```python
from build123d import *

# Parameters (mm, degrees)
BASE_BLOCK_DEPTH         = 25
TOWER_SKETCH_40X40_W     = 40
TOWER_SKETCH_40X40_H     = 40
TOWER_BLOCK_DEPTH        = 55
RIDGE_SADDLE_BODY_DEPTH  = 25
RIDGE_FILLET_R3_R        = 3
SADDLE_OPENING_CUT_DEPTH = 90.022469074
RIDGE_GROOVE_CUT_DEPTH   = 99.994949366
EDGE_FILLET_R5_R         = 5


with BuildPart() as part:
    # Base Profile Sketch → Base Block (new body)
    with BuildSketch(Plane(origin=(0, 0, 0), x_dir=(0, 0, -1), z_dir=(1, 0, 0))):
        with BuildLine():
            Line((-17.320508076, -10), (-25, -10))
            Line((-25, -10), (-25, -20))
            Line((-25, -20), (-12, -20))
            Line((-12, -20), (-12, 0))
            ThreePointArc((-12, 0), (0, 12), (12, 0))
            Line((12, 0), (12, -20))
            Line((12, -20), (25, -20))
            Line((25, -20), (25, -10))
            Line((25, -10), (17.320508076, -10))
            ThreePointArc((17.320508076, -10), (0, 20), (-17.320508076, -10))
        make_face()
    extrude(amount=-BASE_BLOCK_DEPTH)

    # Tower Sketch 40x40 → Tower Block (add)
    with BuildSketch(Plane.ZY.offset(25)):
        Rectangle(TOWER_SKETCH_40X40_W, TOWER_SKETCH_40X40_H)
    extrude(amount=TOWER_BLOCK_DEPTH)

    # Ridge Profile Sketch → Ridge Saddle Body (add, symmetric)
    with BuildSketch(Plane.XY):
        Polygon((-80, -4.997409114), (-30.018519933, 30), (-24.56, 30), (-10.001190629, -10), (0, -10), (0, -20), (-80, -20), align=None)
    extrude(amount=RIDGE_SADDLE_BODY_DEPTH, both=True)

    # Ridge Fillet R3
    ridge_fillet_r3_edges = [part.edges().sort_by_distance(p)[0] for p in [
        (-30.018519933, 30, 0),
        (-24.56, 30, 0),
    ]]
    fillet(ridge_fillet_r3_edges, radius=RIDGE_FILLET_R3_R)

    # Saddle Opening Sketch → Saddle Opening Cut (cut, through all)
    with BuildSketch(Plane(origin=(0, 0, 0), x_dir=(0, 0, -1), z_dir=(1, 0, 0))):
        with BuildLine():
            Line((12, 0), (12, -10))
            Line((12, -10), (12, -20))
            Line((12, -20), (-12, -20))
            Line((-12, -20), (-12, -10))
            Line((-12, -10), (-12, 0))
            ThreePointArc((-12, 0), (0, 12), (12, 0))
        make_face()
    extrude(amount=-SADDLE_OPENING_CUT_DEPTH, mode=Mode.SUBTRACT)

    # Ridge Groove Sketch → Ridge Groove Cut (cut, through all)
    with BuildSketch(Plane.XY.offset(25)):
        with BuildLine():
            Line((-50, -20), (-20, -20))
            ThreePointArc((-20, -20), (-35, -5), (-50, -20))
        make_face()
    extrude(amount=-RIDGE_GROOVE_CUT_DEPTH, mode=Mode.SUBTRACT)

    # Edge Fillet R5
    edge_fillet_r5_edges = [part.edges().sort_by_distance(p)[0] for p in [
        (-10.001190629, -10, -21.160254038),
        (-10.001190629, -10, 21.160254038),
    ]]
    fillet(edge_fillet_r5_edges, radius=EDGE_FILLET_R5_R)


solid = part.part
```
Input: part model. Units: mm. Frame: model coordinates. A direction names the side the tool comes from. Round coordinates to 2 decimals unless told otherwise and drop trailing zeros. Order: outer loops, then holes, each group sorted by start corner. A loop starts at its lowest first (then second) coordinate and runs counter-clockwise, first axis right, second up. Notation, with made-up numbers: (29.25, 60.5) - (77.25, 60.5) arc R9 ccw to (77.25, 67.5) - close; hole circle Ø9 at (13, -13.75). An arc over 180 degrees is marked (long way). One line per question, with ' | ' between items. Start each with the question number.
1) Ray query, probe 1 along Z at (x, y) = (-54, -12); probe 2 along Z at (x, y) = (-73.5, 19.5); probe 3 along Z at (x, y) = (-5, -6). Return the intervals inside material, ascending.
2) Cut plane C-C, the plane x = -35. Return the cut outline in (y, z), then the cut area to 3 significant figures.
3) Cut plane D-D, the plane y = 13.5. Return the cut outline in (x, z).
4) Pull-direction query (X, two-part tool) for faces 6 (the cylindrical face through (-35, -5, -18)), 7 (the cylindrical face through (-9.33, -9.12, 21.11)), 8 (the flat face through (-70, 13, 20)); classes: +X half, -X half, draft (parallel to the pull), parting line (faces both ways), or undercut.
5) Cut plane A-A, the plane y = -11.5. Return the cut outline in (x, z).
6) Cut plane B-B, the plane z = 0. Return the cut outline in (x, y), then the cut area to 3 significant figures.
7) Contact query for flat-ended pins moving along their axis: P1, Ø3.5, axis at x = -2.5, z = 20, coming from the +Y side; P2, Ø5, axis at x = -20.5, z = 12, coming from the -Y side; P3, Ø1.5, axis at x = -61, z = -9.5, coming from the -Y side; P4, Ø10.5, axis at x = -66, z = 6, coming from the +Y side. Output: stop coordinate, or through.
8) Set-up query: faces 1 (the cylindrical face through (-8.1, 19.99, -0.59)), 2 (the flat face through (-62, 20, 0)), 3 (the cylindrical face through (-9.403, -9.071, -21.214)), 4 (the flat face through (-70, 13, -20)), 5 (the flat face through (-39, -5, -12)). Return all of +Z, -Z, +X, -X, +Y, -Y with unobstructed straight access to the full face (end or side cutting, diameter ignored); none if empty.
Worked out:
1) probe 1: z = -25 to -12, 12 to 25 | probe 2: z = -20 to 20 | probe 3: z = -19.08 to -12, 12 to 19.08
2) outline: (-5, -25) - (26.51, -25) - (26.51, 25) - (-5, 25) - (-5, 12) - (0, 12) arc R12 cw to (0, -12) - (-5, -12) - close | area: 1,230 mm^2
3) outline: (-80, -20) - (-53.58, -20) - (-53.58, -25) - (-18.55, -25) - (-18.55, -14.76) - (0, -14.76) - (0, 14.76) - (-18.55, 14.76) - (-18.55, 25) - (-53.58, 25) - (-53.58, 20) - (-80, 20) - close
4) face 6: undercut | face 7: +X half | face 8: draft
5) outline: (-80, -25) - (-47.36, -25) - (-47.36, -12) - (-80, -12) - close; (-80, 12) - (-47.36, 12) - (-47.36, 25) - (-80, 25) - close; (-22.64, -25) - (0, -25) - (0, -12) - (-22.64, -12) - close; (-22.64, 12) - (0, 12) - (0, 25) - (-22.64, 25) - close
6) outline: (-80, 12) - (0, 12) - (0, 20) - (-20.92, 20) - (-23.84, 28.03) arc R3 ccw to (-26.66, 30) - (-29.07, 30) arc R3 ccw to (-30.79, 29.46) - (-44.3, 20) - (-80, 20) - close | area: 783 mm^2
7) P1: stops at y = 8.18 | P2: stops at y = -20 | P3: stops at y = 6.24 | P4: stops at y = 20
8) face 1: +X | face 2: +Z, -Z, -X, +Y | face 3: -Z, +X | face 4: -Z, -X, +Y | face 5: +X, -X, -Y
